Read the model definition and answer for the solid it produces. Units are mm, in the model's axes. A direction names the side the tool comes from. Give positions to 0.01 mm unless a question says otherwise; leave off trailing zeros. Loops run counter-clockwise (first coordinate to the right, second up) from the corner with the lowest first, then second, coordinate; pieces in that order, holes last. Notation, with made-up numbers: (89.25, 78) - (94.25, 78) arc R5 ccw to (94.25, 86) - close; hole circle Ø3 at (87, -16). An arc over 180 degrees is marked (long way). Put each result on its own line as item: value. Start each with the question number.
1. Given pin 1 Ø1.5 at (x, y) = (6, 5.5) entering from -Z; pin 2 Ø4 at (y, z) = (7, -15.5) entering from +X; pin 3 Ø2 at (x, y) = (-19.5, 6) entering from +Z, each flat-ended and moving along its own axis, determine where each tip first touches the part or whether it passes through.
2. For a pull along Z with two mould halves and no side action, classify faces 3 (the cylindrical face through (-21.58, 6.9, -6.8)), 4 (the flat face through (-16, 2, 26)), 5 (the cylindrical face through (21, 7, 28)) as released by +Z, released by -Z, zero draft, split by the parting line, or undercut.
3. A cutting plane is placed at C-C, the plane y = 9.5. Determine the outline of the cut face in (x, z) (3 decimals), plus the area to 3 significant figures.
4. A cutting plane is placed at B-B, the plane x = 0. Determine the outline of the cut face in (y, z) (3 decimals), plus the area to 4 significant figures.
5. For faces 1 (the cylindrical face through (-1.32, 1.01, 29.97)), 2 (the flat face through (22, 14, 8)), determine the directions among +Z, -Z, +X, -X, +Y, -Y from which every point of the face is accessible in a straight line to the end or side of a thin tool.
6. A cutting plane is placed at A-A, the plane z = 0. Determine the outline of the cut face in (x, y) (3 decimals), plus the area to 4 significant figures.
7. Consider L1, parallel to Z at x = 0, y = 8.25 (3 decimals); L2, parallel to X at y = 4.5, z = -5; L3, parallel to X at y = 9, z = -6.5. Determine where each line is inside the solid, lowest interval first. Write a range as from..to.
```python
from build123d import *

# Parameters (mm, degrees)
G1_1_2_TAPPED_HOLE1_D     = 45.25
G1_1_2_TAPPED_HOLE1_DEPTH = 102.54
G1_1_2_TAPPED_HOLE1_TIP   = 13.594471505


with BuildPart() as part:
    # Sketch1 → Revolve1 (revolve)
    with BuildSketch(Plane(origin=(0, 0, 0), x_dir=(0, 0, -1), z_dir=(1, 0, 0))):
        Polygon((35, 12), (33, 14), (22.5, 14), (22.5, 0), (30, 0), (30, 2), (35, 2), align=None)
    revolve(axis=Axis((0, 0, 0), (0, 1, 0)))

    # G1-1/2 Tapped Hole1
    with Locations(Plane(origin=(0, 14, 0), x_dir=(1, 0, 0), z_dir=(0, 1, 0))):
        with Locations((0, 0)):
            Hole(G1_1_2_TAPPED_HOLE1_D / 2, depth=G1_1_2_TAPPED_HOLE1_DEPTH)
            with Locations((0, 0, -(G1_1_2_TAPPED_HOLE1_DEPTH + G1_1_2_TAPPED_HOLE1_TIP / 2))):  # 118° drill point
                Cone(0, G1_1_2_TAPPED_HOLE1_D / 2, G1_1_2_TAPPED_HOLE1_TIP, mode=Mode.SUBTRACT)


solid = part.part
```
Return value:
1. pin 1: stops at z = -34.6
1. pin 2: stops at x = 32.29
1. pin 3: stops at z = 29.71
2. face 3: undercut
2. face 4: zero draft
2. face 5: split by the parting line
3. outline: circle Ø70 at (0, 0); hole circle Ø45.25 at (0, 0)
3. area: 2,240 mm2
4. outline: (0, -30) - (2, -30) - (2, -35) - (12, -35) - (14, -33) - (14, -22.625) - (0, -22.625) - close; (0, 22.625) - (14, 22.625) - (14, 33) - (12, 35) - (2, 35) - (2, 30) - (0, 30) - close
4. area: 322.5 mm2
5. face 1: -Y
5. face 2: +Z, -Z, +X, -X, +Y
6. outline: (-35, 2) - (-30, 2) - (-30, 0) - (-22.625, 0) - (-22.625, 14) - (-33, 14) - (-35, 12) - close; (22.625, 0) - (30, 0) - (30, 2) - (35, 2) - (35, 12) - (33, 14) - (22.625, 14) - close
6. area: 322.5 mm2
7. L1: z = -35..-22.625, 22.625..35
7. L2: x = -34.64..-22.07, 22.07..34.64
7. L3: x = -34.39..-21.67, 21.67..34.39
